```python
from build123d import *

# Parameters (mm, degrees)
EXTRUDE_419_DEPTH = 6.4
FILLET_1345_R     = 0.4


with BuildPart() as part:
    # 草图1 → Extrude 419 (new body)
    with BuildSketch(Plane(origin=(0, 0, 0), x_dir=(0, 0, -1), z_dir=(1, 0, 0))):
        Polygon((8, 4.618802154), (8, -4.618802154), (0, -9.237604307), (-8, -4.618802154), (-8, 4.618802154), (0, 9.237604307), align=None)
    extrude(amount=EXTRUDE_419_DEPTH)

    # 草图2 → 凸台-旋转1 (revolve)
    with BuildSketch(Plane.XY, mode=Mode.PRIVATE) as revolve_1_sk:
        Polygon((0, 0), (51.4, 0), (51.4, 4.134), (51.4, 5), (25.7, 5), (0, 5), align=None)
    revolve(revolve_1_sk.sketch.rotate(Axis((0, 0, 0), (1, 0, 0)), 90), axis=Axis((0, 0, 0), (1, 0, 0)))

    # 草图3 → 切除-旋转1 (revolve, cut)
    with BuildSketch(Plane.XY):
        Polygon((0, 8), (3.601282526, 14.237604307), (3.601282526, 19.237604307), (-10, 19.237604307), (-10, 8), align=None)
    revolve(axis=Axis((0, 0, 0), (1, 0, 0)), mode=Mode.SUBTRACT)

    # 草图4 → 切除-旋转3 (revolve, cut)
    with BuildSketch(Plane.XY, mode=Mode.PRIVATE) as cut_revolve_3_sk:
        Polygon((6.4, 7.315), (5.8, 7.661410162), (5.8, 9.237604307), (6.4, 9.237604307), align=None)
    revolve(cut_revolve_3_sk.sketch.rotate(Axis((0, 0, 0), (1, 0, 0)), 90), axis=Axis((0, 0, 0), (1, 0, 0)), mode=Mode.SUBTRACT)

    # Fillet 1345
    fillet_1345_edges = [part.edges().sort_by_distance(p)[0] for p in [
        (6.4, 0, -5),
    ]]
    fillet(fillet_1345_edges, radius=FILLET_1345_R)

    # 草图6 → 切除-旋转4 (revolve, cut)
    with BuildSketch(Plane.XY, mode=Mode.PRIVATE) as cut_revolve_4_sk:
        Polygon((50.9, 5), (51.9, 5), (51.4, 4.133974596), align=None)
    revolve(cut_revolve_4_sk.sketch.rotate(Axis((0, 0, 0), (1, 0, 0)), 90), axis=Axis((0, 0, 0), (1, 0, 0)), mode=Mode.SUBTRACT)


solid = part.part
```
CAD build for the part. Positions are in the model's coordinates, mm. A direction names the side the tool comes from. Coordinates: 2 decimals unless noted, no trailing zeros. Loops run counter-clockwise (first coordinate to the right, second up) from the corner with the lowest first, then second, coordinate; pieces in that order, holes last. Notation, with made-up numbers: (76.5, -20) - (114.5, -20) arc R34 ccw to (114.5, 17) - close; hole circle Ø5 at (-27.5, 54). An arc over 180 degrees is marked (long way). Return JSON: item names as keys, results as strings.
1. Probe L1, parallel to Z at x = 13, y = 3; L2, parallel to X at y = 5.5, z = 2; L3, parallel to Y at x = 23, z = 0.25. List the from-to ranges inside material, lowest first. Write a range as from..to.
Result:
{"L1": "z = -4..4", "L2": "x = 0..6.4", "L3": "y = -4.99..4.99"}
2. Drop flat-ended pins along their axis: pin 1 (2 mm diameter, centred on x = 37, y = -7.5, fed in from +Z); pin 2 (8 mm diameter, centred on x = 19.5, z = -1, fed in from -Y); pin 3 (10 mm diameter, centred on x = 39.5, y = -6, fed in from +Z); pin 4 (10 mm diameter, centred on x = 31, y = -0.5, fed in from +Z). Give the stop position or say it passes through.
Result:
{"pin 1": "passes through", "pin 2": "stops at y = -5", "pin 3": "stops at z = 4.9", "pin 4": "stops at z = 5"}
3. Band-saw the part on A-A (x = 45.5). Give the cut face in (y, z), and give its area (3 significant figures).
Result:
{"outline": "circle Ø10 at (0, 0)", "area": "78.5 mm2"}
4. 3-axis set-ups, long thin cutter, end or side, ignore diameter. For faces 1 (the cylindrical face through (29, 0, -5)), 2 (the flat face through (2.859, 6.961, -3.944)): which of +Z, -Z, +X, -X, +Y, -Y reach the whole face in a straight line?
Result:
{"face 1": "+X", "face 2": "-Z, +X, -X, +Y"}
